Source: CAD feature listing. Evaluate the final solid. Frame: model axes, mm. A direction names the side the tool comes from. Give positions to 0.01 mm unless a question says otherwise; leave off trailing zeros. Write each loop counter-clockwise with the first axis right and the second up, starting at its lowest first coordinate (ties: lowest second). Pieces come first, ordered by that corner, then holes. Notation, with made-up numbers: (-19, 57.5) -> (0, 57.5) arc R10 ccw to (0, 65.5) -> close; hole circle Ø9 at (-16, 20.25). An arc over 180 degrees is marked (long way). Write item = value, one per line.
from build123d import *

# Parameters (mm, degrees)
SKETCH1_R           = 25
BOSS_EXTRUDE1_DEPTH = 180
SKETCH2_R           = 15
BOSS_EXTRUDE2_DEPTH = 90
CUT_EXTRUDE1_START  = -20
CUT_EXTRUDE1_DEPTH  = 120
CHAMFER1_SIZE       = 1
CUT_EXTRUDE2_START  = -10
SKETCH4_R           = 2.5
CUT_EXTRUDE2_DEPTH  = 10


with BuildPart() as part:
    # Sketch1 → Boss-Extrude1 (new body)
    with BuildSketch(Plane.XY):
        with Locations(Location((0, 0, 0), (0, 0, 180))):
            Circle(SKETCH1_R)
    extrude(amount=BOSS_EXTRUDE1_DEPTH)

    # Sketch2 → Boss-Extrude2 (add)
    with BuildSketch(Plane.XY.offset(180)):
        with Locations(Location((0, 0, 0), (0, 0, 180))):
            Circle(SKETCH2_R)
    extrude(amount=BOSS_EXTRUDE2_DEPTH)

    # Sketch3 → Cut-Extrude1 (cut)
    with BuildSketch(Plane(origin=(0, 0, 0), x_dir=(1, 0, 0), z_dir=(0, 1, 0)).offset(CUT_EXTRUDE1_START)):
        with BuildLine():
            Line((6, -84.229937471), (6, -134.229937471))
            ThreePointArc((6, -134.229937471), (0, -140.229937471), (-6, -134.229937471))
            Line((-6, -134.229937471), (-6, -84.229937471))
            ThreePointArc((-6, -84.229937471), (0, -78.229937471), (6, -84.229937471))
        make_face()
    extrude(amount=-CUT_EXTRUDE1_DEPTH, mode=Mode.SUBTRACT)

    # Chamfer1
    chamfer1_edges = [part.edges().sort_by_distance(p)[0] for p in [
        (25, 0, 0),
        (25, 0, 180),
        (15, 0, 270),
    ]]
    chamfer(chamfer1_edges, length=CHAMFER1_SIZE)

    # Sketch4 → Cut-Extrude2 (cut)
    with BuildSketch(Plane(origin=(0, 0, 0), x_dir=(0, 0, -1), z_dir=(1, 0, 0)).offset(CUT_EXTRUDE2_START)):
        with Locations((-211, 0)):
            Circle(SKETCH4_R)
    extrude(amount=-CUT_EXTRUDE2_DEPTH, mode=Mode.SUBTRACT)


solid = part.part
1) Cut plane D-D (z = 122.5). Return the cut outline in (x, y), then the cut area to 3 significant figures.
Computed:
outline = (-6, -24.27) -> (-6, -20) -> (6, -20) -> (6, -24.27) arc R25 ccw (long way) to start
area = 1,910 mm²
2) Cut plane C-C (z = 163.5). Return the cut outline in (x, y).
Computed:
outline = circle Ø50 at (0, 0)
3) Material intervals for L1, parallel to Z at x = 16, y = 0.5; L2, parallel to Y at x = -11, z = 211; L3, parallel to Y at x = -11.65, z = 211, sorted ascending.
Computed:
L1 = 0 to 180
L2 = -10.2 to -2.5, 2.5 to 10.2
L3 = -9.45 to -2.5, 2.5 to 9.45
4) Cut plane A-A (x = 0). Return the cut outline in (y, z), then the cut area to 3 significant figures.
Computed:
outline = (-25, 1) -> (-24, 0) -> (24, 0) -> (25, 1) -> (25, 179) -> (24, 180) -> (15, 180) -> (15, 269) -> (14, 270) -> (-14, 270) -> (-15, 269) -> (-15, 180) -> (-24, 180) -> (-25, 179) -> (-25, 140.23) -> (-20, 140.23) -> (-20, 78.23) -> (-25, 78.23) -> close
area = 11,400 mm²
5) Draft query along Z for faces 1 (the cylindrical face through (-11.5, 22.2, 88.8)), 2 (the flat face through (0, 16, 180)), 3 (the flat face through (6, -22, 109)). Return one class per face: pulls with the +Z half, pulls with the -Z half, needs draft (parallel to the pull), parting line crosses it, or undercut.
Computed:
face_1 = needs draft
face_2 = pulls with the +Z half
face_3 = undercut
6) Contact query for flat-ended pins moving along their axis: pin 1 (3 mm diameter, centred on x = 11.5, z = 225, fed in from -Y); pin 2 (2.5 mm diameter, centred on y = -1, z = 210.5, fed in from -X); pin 3 (6 mm diameter, centred on x = -3.5, z = 97, fed in from -Y); pin 4 (12 mm diameter, centred on y = 3, z = 89, fed in from -X). Output: stop coordinate, or through.
Computed:
pin_1 = -11.18
pin_2 = -10
pin_3 = -24.27
pin_4 = -25
7) Access query for faces 4 (the cylindrical face through (0.13, -22.47, 140.23)), 5 (the cylindrical face through (-8.06, -12.65, 223.88)), 6 (the flat face through (-10, 0, 211)), 7 (the flat face through (0, 0, 0)). Directions: +Z, -Z, +X, -X, +Y, -Y. A direction counts if a zero-diameter tool reaches every point of the face in a straight line with its end or side. Return the directions, or none.
Computed:
face_4 = -Y
face_5 = +Z
face_6 = -X
face_7 = -Z, +X, -X, +Y, -Y
8) Cut plane B-B (y = 0). Return the cut outline in (x, z), then the cut area to 3 significant figures.
Computed:
outline = (-25, 1) -> (-24, 0) -> (24, 0) -> (25, 1) -> (25, 179) -> (24, 180) -> (15, 180) -> (15, 269) -> (14, 270) -> (-14, 270) -> (-15, 269) -> (-15, 213.5) -> (-10, 213.5) -> (-10, 208.5) -> (-15, 208.5) -> (-15, 180) -> (-24, 180) -> (-25, 179) -> close
area = 11,700 mm²
